Verification items for this drawing (mm, ordinates from the low corner). Round coordinates to 2 decimals unless told otherwise and drop trailing zeros. Write each loop counter-clockwise with the first axis right and the second up, starting at its lowest first coordinate (ties: lowest second). Pieces come first, ordered by that corner, then holes. Notation, with made-up numbers: (-5.75, 65) -> (0.25, 65) arc R6 ccw to (0.25, 71) -> close; hole circle Ø5 at (-20, 83). An arc over 180 degrees is marked (long way). Put each result on its own line as item: value. Start each with the question number.
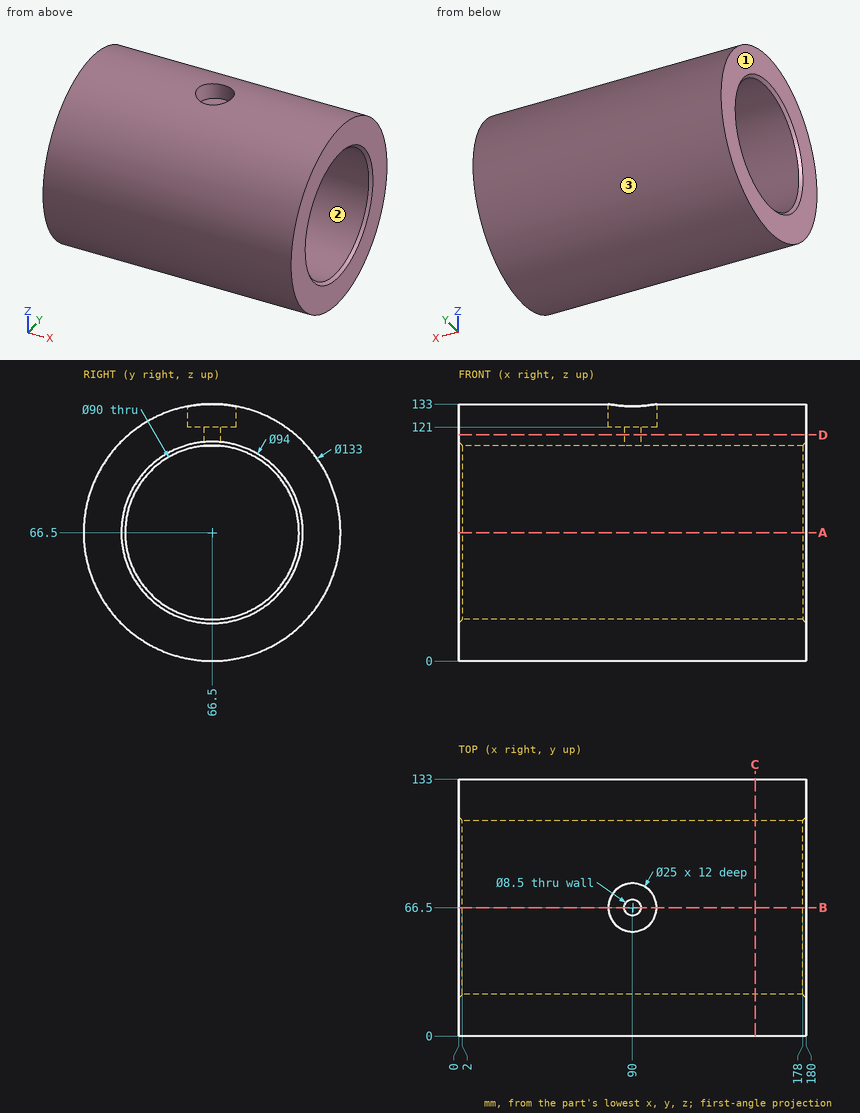
1. Section check D-D, the plane z = 117. Enter the section's corners in (x, y), then the cut area to 3 significant figures.
2. Draft check along Y on the marked faces 1, 2 and 3. Enter one of: released by +Y, released by -Y, zero draft, split by the parting line, or undercut.
3. Section check A-A, the plane z = 66.5. Enter the section's corners in (x, y).
4. Gauge pin test, flat ends, axial feed: P1, Ø12, axis at x = 50.5, z = 118, coming from the +Y side; P2, Ø2, axis at x = 149, y = 95, coming from the -Z side; P3, Ø3, axis at x = 110.5, y = 14.5, coming from the -Z side; P4, Ø10, axis at x = 34, y = 69, coming from the +Z side. Record the tip position at first contact, or that the pin passes through.
5. Section check C-C, the plane x = 153.5. Enter the section's corners in (y, z), then the cut area to 3 significant figures.
6. Material ranges on L1, parallel to X at y = 66, z = 125; L2, parallel to Y at x = 90, z = 113.5; L3, parallel to Y at x = 142, z = 66.5, recorded low to high. Write a range as [from, to].
7. Section check B-B, the plane y = 66.5. Enter the section's corners in (x, z).
Reply:
1. outline: (0, 23.23) -> (180, 23.23) -> (180, 109.77) -> (0, 109.77) -> close; hole circle Ø8.5 at (90, 66.5)
1. area: 15,500 mm2
2. face 1: zero draft
2. face 2: undercut
2. face 3: split by the parting line
3. outline: (0, 0) -> (180, 0) -> (180, 19.5) -> (178, 21.5) -> (2, 21.5) -> (0, 19.5) -> close; (0, 113.5) -> (2, 111.5) -> (178, 111.5) -> (180, 113.5) -> (180, 133) -> (0, 133) -> close
4. P1: stops at y = 115
4. P2: stops at z = 5.95
4. P3: stops at z = 23.23
4. P4: stops at z = 133
5. outline: circle Ø133 at (66.5, 66.5); hole circle Ø90 at (66.5, 66.5)
5. area: 7,530 mm2
6. L1: x = [0, 77.51], [102.49, 180]
6. L2: y = [19.45, 62.25], [70.75, 113.55]
6. L3: y = [0, 21.5], [111.5, 133]
7. outline: (0, 0) -> (180, 0) -> (180, 19.5) -> (178, 21.5) -> (2, 21.5) -> (0, 19.5) -> close; (0, 113.5) -> (2, 111.5) -> (85.75, 111.5) -> (85.75, 121) -> (77.5, 121) -> (77.5, 133) -> (0, 133) -> close; (94.25, 111.5) -> (178, 111.5) -> (180, 113.5) -> (180, 133) -> (102.5, 133) -> (102.5, 121) -> (94.25, 121) -> close
